```python
from build123d import *

# Parameters (mm, degrees)
BOSS_EXTRUDE1_DEPTH = 40
SHELL1_T            = -5


with BuildPart() as part:
    # Sketch1 → Boss-Extrude1 (new body)
    with BuildSketch(Plane.XY):
        with BuildLine():
            Line((-11.59263729, -51.941945741), (92.170688637, -51.941945741))
            Line((92.170688637, -51.941945741), (123.739238561, -51.941945741))
            Line((123.739238561, -51.941945741), (123.739238561, 120.781051565))
            ThreePointArc((123.739238561, 120.781051565), (117.881374185, 134.923187188), (103.739238561, 140.781051565))
            Line((103.739238561, 140.781051565), (8.40736271, 140.781051565))
            ThreePointArc((8.40736271, 140.781051565), (-5.734772914, 134.923187188), (-11.59263729, 120.781051565))
            Line((-11.59263729, 120.781051565), (-11.59263729, -51.941945741))
        make_face()
    extrude(amount=BOSS_EXTRUDE1_DEPTH)

    # Shell1
    shell1_openings = [part.faces().sort_by_distance(p)[0] for p in [
        (56.073300636, 43.810653181, 0),
    ]]
    offset(amount=SHELL1_T, openings=shell1_openings, kind=Kind.INTERSECTION)


solid = part.part
```
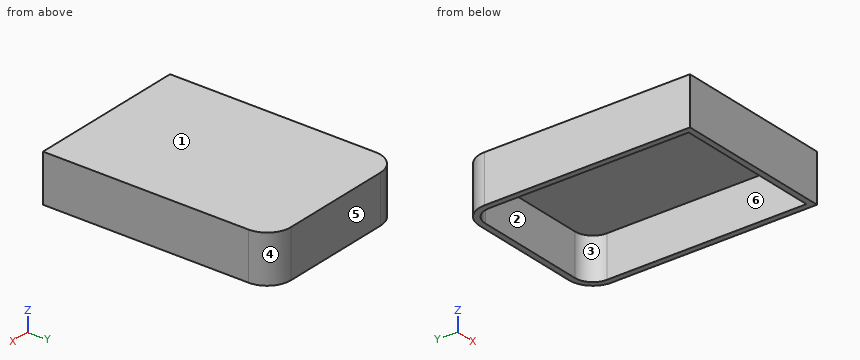
The model under review builds one solid part; all positions refer to its coordinate system, in mm. Face numbers are marked on the shaded views. A direction names the side the tool comes from. Give positions to 0.01 mm unless a question says otherwise; leave off trailing zeros. Write each loop counter-clockwise with the first axis right and the second up, starting at its lowest first coordinate (ties: lowest second). Pieces come first, ordered by that corner, then holes. Notation, with made-up numbers: M -17.5,-30 L 11.5,-30 A25 cw 11.5,-18 Z; hole C 88,76 d6. An arc over 180 degrees is marked long. Write each question's results on one line, items separated by ' | '. Start each with the question number.
1. We need section A-A (y = -23). Write out the cut boundary in (x, z), and give its area (3 significant figures).
2. For the marked faces 5 and 6, list the 3-axis set-ups (+Z, -Z, +X, -X, +Y, -Y) from which the entire face can be reached by the end or side of a thin tool; tool diameter is ignored.
3. Insertion check: pin 1 Ø2 at (x, y) = (31.5, 89) entering from -Z; pin 2 Ø6 at (x, z) = (3, 21) entering from +Y. Each pin has a flat end and moves straight along its axis. Give the tip position at first contact, or say it passes through.
4. For probe 1 along Y at (x, z) = (27.5, 27.5); probe 2 along X at (y, z) = (82.5, 10); probe 3 along Z at (x, y) = (47.5, 60), list the stretches that pass through material, from the lowest coordinate up. Write a range as [from, to].
5. We need section C-C (x = 57.5). Write out the cut boundary in (y, z), and give its area (3 significant figures).
6. We need section B-B (z = 30). Write out the cut boundary in (x, y).
7. Mouldability with a two-part tool opening along Y and no side actions: class the marked faces 1, 2, 3 and 4 as released by +Y, released by -Y, zero draft, split by the parting line, or undercut.
Results found:
1) outline: M -11.59,0 L -6.59,0 L -6.59,35 L 118.74,35 L 118.74,0 L 123.74,0 L 123.74,40 L -11.59,40 Z | area: 1,030 mm^2
2) face 5: +Z, -Z, +X, -X, +Y | face 6: -Z
3) pin 1: stops at z = 35 | pin 2: stops at y = 140.64
4) probe 1: y = [-51.94, -46.94], [135.78, 140.78] | probe 2: x = [-11.59, -6.59], [118.74, 123.74] | probe 3: z = [35, 40]
5) outline: M -51.94,0 L -46.94,0 L -46.94,35 L 135.78,35 L 135.78,0 L 140.78,0 L 140.78,40 L -51.94,40 Z | area: 1,310 mm^2
6) outline: M -11.59,-51.94 L 123.74,-51.94 L 123.74,120.78 A20 ccw 103.74,140.78 L 8.41,140.78 A20 ccw -11.59,120.78 Z; hole M -6.59,-46.94 L 118.74,-46.94 L 118.74,120.78 A15 ccw 103.74,135.78 L 8.41,135.78 A15 ccw -6.59,120.78 Z
7) face 1: zero draft | face 2: undercut | face 3: undercut | face 4: released by +Y
